Job drawing, mm, ordinate dimensions from the low corner. One solid piece. A direction names the side the tool comes from. Round coordinates to 2 decimals unless told otherwise and drop trailing zeros. Write each loop counter-clockwise with the first axis right and the second up, starting at its lowest first coordinate (ties: lowest second). Pieces come first, ordered by that corner, then holes. Notation, with made-up numbers: M -23.75,11 L 11.25,11 A29 cw 11.25,38 Z; hole C 1.5,21 d4. An arc over 180 degrees is marked long. Write each question's results on one line, items separated by ' | '. Start each with the question number.
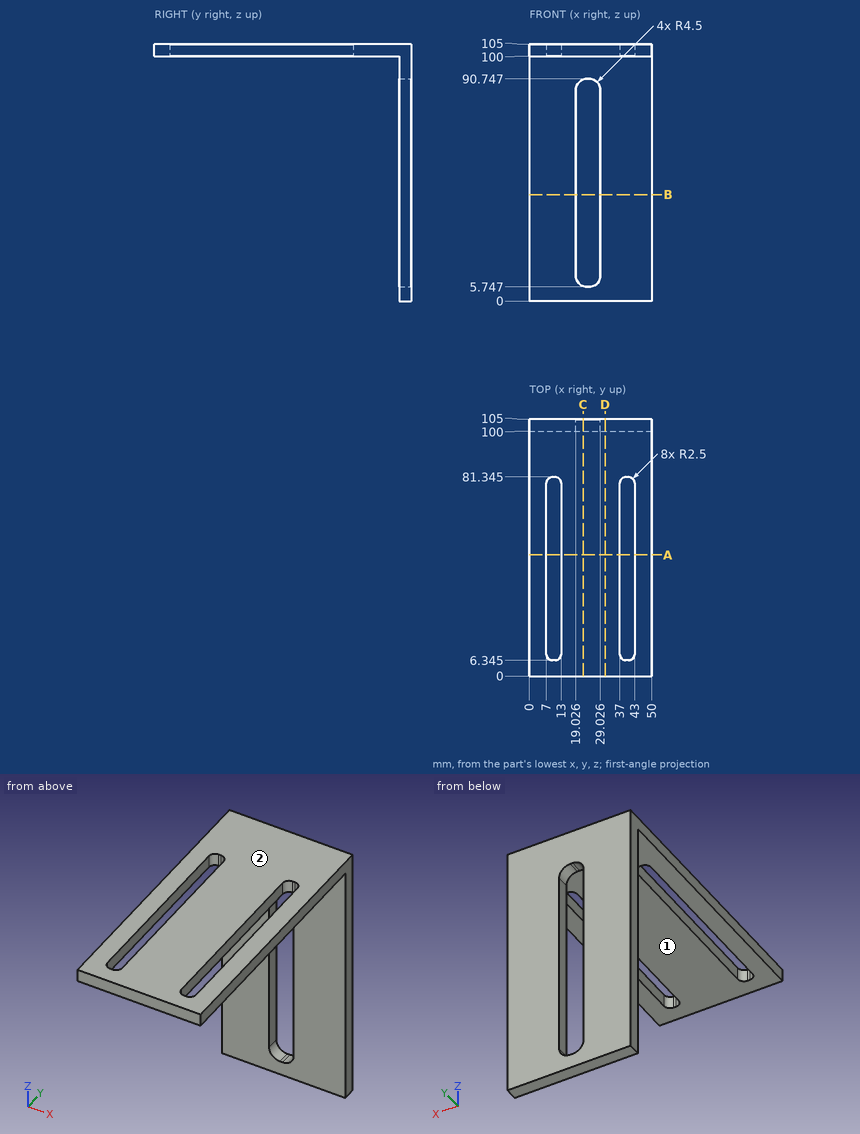
1) Wall check: line 1 along Y through (x, z) = (10, 11.5). Give the ranges that are in metal, low to high. Write a range as from..to.
2) Saw through at D-D, the plane x = 31. Write the cut outline in (y, z), plus the area to 4 significant figures.
3) Drop flat-ended pins along their axis: pin 1 Ø8 at (x, z) = (21.5, 25) entering from +Y; pin 2 Ø1.5 at (x, z) = (12, 13) entering from -Y; pin 3 Ø15 at (x, y) = (31, 61) entering from -Z; pin 4 Ø1 at (x, y) = (9, 27.5) entering from +Z. Give the stop position or say it passes through.
4) Saw through at A-A, the plane y = 49.5. Write the cut outline in (x, z).
5) 3-axis set-ups, long thin cutter, end or side, ignore diameter. For the marked faces 1 and 2: which of +Z, -Z, +X, -X, +Y, -Y reach the whole face in a straight line?
6) Saw through at C-C, the plane x = 22. Write the cut outline in (y, z), plus the area to 3 significant figures.
7) Saw through at B-B, the plane z = 43.5. Write the cut outline in (x, y).
Filled sheet:
1) line 1: y = 100..105
2) outline: M 0,100 L 100,100 L 100,0 L 105,0 L 105,105 L 0,105 Z | area: 1,025 mm^2
3) pin 1: stops at y = 105 | pin 2: stops at y = 100 | pin 3: stops at z = 100 | pin 4: passes through
4) outline: M 0,100 L 7,100 L 7,105 L 0,105 Z; M 13,100 L 37,100 L 37,105 L 13,105 Z; M 43,100 L 50,100 L 50,105 L 43,105 Z
5) face 1: -Z, +X, -X, -Y | face 2: +Z, +X, -X, +Y, -Y
6) outline: M 0,100 L 100,100 L 100,90.48 L 105,90.48 L 105,105 L 0,105 Z; M 100,0 L 105,0 L 105,6.01 L 100,6.01 Z | area: 603 mm^2
7) outline: M 0,100 L 19.03,100 L 19.03,105 L 0,105 Z; M 29.03,100 L 50,100 L 50,105 L 29.03,105 Z
